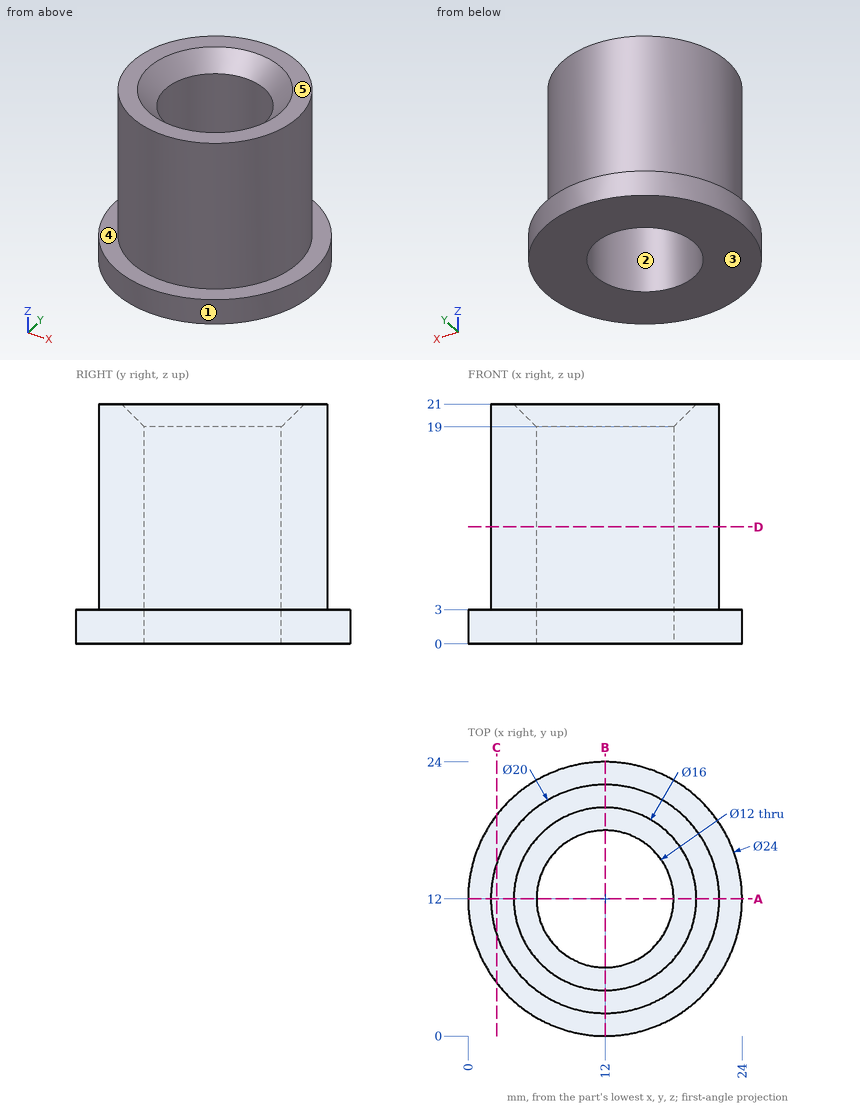
Can you work these out from the drawing? Everything is in mm from the part's minimum corner. A direction names the side the tool comes from. Round coordinates to 2 decimals unless told otherwise and drop trailing zeros. Loops run counter-clockwise (first coordinate to the right, second up) from the corner with the lowest first, then second, coordinate; pieces in that order, holes last. Notation, with made-up numbers: M 21.25,19 L 39.25,19 A15 ccw 39.25,41 Z; hole C 0.25,66 d2. An arc over 180 degrees is marked long. Answer in a Markdown table with one row per item.
1. If we section it at D-D, the plane z = 10.25: Please give me the cut outline in (x, y).
Established:
| item | result |
|---|---|
| outline | C 12,12 d20; hole C 12,12 d12 |
2. If we section it at C-C, the plane x = 2.5: Please give me the cut outline in (y, z), plus the area to 3 significant figures.
Established:
| item | result |
|---|---|
| outline | M 4.67,0 L 19.33,0 L 19.33,3 L 15.12,3 L 15.12,21 L 8.88,21 L 8.88,3 L 4.67,3 Z |
| area | 156 mm² |
3. I'm going to push flat-ended pins straight in: pin 1 Ø1.5 at (y, z) = (11.5, 17.5) entering from -X; pin 2 Ø2 at (x, z) = (11, 15.5) entering from -Y; pin 3 Ø7 at (x, y) = (9.5, 11) entering from +Z. Where does each tip first touch, or does it pass through?
Established:
| item | result |
|---|---|
| pin 1 | x = 2 |
| pin 2 | y = 2 |
| pin 3 | z = 19.19 |
4. On a 3-axis mill with a long thin cutter (end or side, diameter ignored), from which of +Z, -Z, +X, -X, +Y, -Y can I reach the whole of each face in a straight line? I mean the marked faces 4 and 5. Say none if no direction works.
Established:
| item | result |
|---|---|
| face 4 | +Z |
| face 5 | +Z, +X, -X, +Y, -Y |
5. If we section it at A-A, the plane y = 12: Please give me the cut outline in (x, z), plus the area to 3 significant figures.
Established:
| item | result |
|---|---|
| outline | M 0,0 L 6,0 L 6,19 L 4,21 L 2,21 L 2,3 L 0,3 Z; M 18,0 L 24,0 L 24,3 L 22,3 L 22,21 L 20,21 L 18,19 Z |
| area | 176 mm² |
6. Please list where these lines run through material, in increasing order: line 1 (Y direction, x = 12, z = 12.75); line 2 (Z direction, x = 4.25, y = 4); line 3 (Y direction, x = 13.25, z = 16.5). Write a range as from..to.
Established:
| item | result |
|---|---|
| line 1 | 2..6, 18..22 |
| line 2 | 0..3 |
| line 3 | 2.08..6.13, 17.87..21.92 |
7. Thinking about a two-plate mould opening in Y: for the marked faces 1, 2 and 3, which applies, pulls with the +Y half, pulls with the -Y half, needs draft (parallel to the pull), parting line crosses it, or undercut?
Established:
| item | result |
|---|---|
| face 1 | parting line crosses it |
| face 2 | undercut |
| face 3 | needs draft |
